from build123d import *

# Parameters (mm, degrees)
SKETCH_1_R                = 810
EXTRUDE_1_DEPTH           = 25
SKETCH_2_R                = 730
EXTRUDE_2_DEPTH           = 5
CUT_EXTRUDE_1_REACH       = 1147.906
SKETCH_3_R                = 75
SKETCH_4_R                = 110
CUT_EXTRUDE_2_DEPTH       = 5
HOLE_WIZARD_M8_1_D        = 6.8
HOLE_WIZARD_25_5_25_5_1_D = 26
CUT_EXTRUDE_3_DEPTH       = 1146.905755287
CUT_EXTRUDE_3_DEPTH_BACK  = 1146.905755287
SKETCH_10_OUTSIDE_W       = 2080.244
SKETCH_10_OUTSIDE_H       = 2080.244
SKETCH_10_OUTSIDE_R       = 675
CHAMFER_1_SIZE            = 10


with BuildPart() as part:
    # 草图1 → 凸台-拉伸1 (new body)
    with BuildSketch(Plane(origin=(0, 0, 0), x_dir=(1, 0, 0), z_dir=(0, 1, 0))):
        with Locations(Location((0, 0, 0), (0, 0, 270))):
            Circle(SKETCH_1_R)
    extrude(amount=EXTRUDE_1_DEPTH)

    # 草图2 → 凸台-拉伸2 (add)
    with BuildSketch(Plane(origin=(0, 25, 0), x_dir=(1, 0, 0), z_dir=(0, 1, 0))):
        with Locations(Location((0, 0, 0), (0, 0, 270))):
            Circle(SKETCH_2_R)
    extrude(amount=EXTRUDE_2_DEPTH)

    # 草图3 → 切除-拉伸1 (cut, up to next)
    with BuildSketch(Plane(origin=(0, 30, 0), x_dir=(1, 0, 0), z_dir=(0, 1, 0)), mode=Mode.PRIVATE) as cut_extrude_1_sk1:
        with BuildLine():
            Line((130, 662.363193422), (130, -662.363193422))
            ThreePointArc((130, -662.363193422), (521.236510617, -428.879353665), (675, 0))
            ThreePointArc((675, 0), (521.236510617, 428.879353665), (130, 662.363193422))
        make_face()
    cut_extrude_1_tool1 = extrude(cut_extrude_1_sk1.sketch, amount=-CUT_EXTRUDE_1_REACH, mode=Mode.PRIVATE) & part.part
    # 草图3 → 切除-拉伸1 (cut, up to next)
    with BuildSketch(Plane(origin=(0, 30, 0), x_dir=(1, 0, 0), z_dir=(0, 1, 0)), mode=Mode.PRIVATE) as cut_extrude_1_sk2:
        with BuildLine():
            ThreePointArc((-130, 662.363193422), (-675, 0), (-130, -662.363193422))
            Line((-130, -662.363193422), (-130, 662.363193422))
        make_face()
    cut_extrude_1_tool2 = extrude(cut_extrude_1_sk2.sketch, amount=-CUT_EXTRUDE_1_REACH, mode=Mode.PRIVATE) & part.part
    # 草图3 → 切除-拉伸1 (cut, up to next)
    with BuildSketch(Plane(origin=(0, 30, 0), x_dir=(1, 0, 0), z_dir=(0, 1, 0)), mode=Mode.PRIVATE) as cut_extrude_1_sk3:
        with Locations(Location((0, 0, 0), (0, 0, 270))):
            Circle(SKETCH_3_R)
    cut_extrude_1_tool3 = extrude(cut_extrude_1_sk3.sketch, amount=-CUT_EXTRUDE_1_REACH, mode=Mode.PRIVATE) & part.part
    add(cut_extrude_1_tool1.solids().sort_by_distance((357.907844, 30, 0))[0], mode=Mode.SUBTRACT)
    add(cut_extrude_1_tool2.solids().sort_by_distance((-357.907844, 30, 0))[0], mode=Mode.SUBTRACT)
    add(cut_extrude_1_tool3.solids().sort_by_distance((0, 30, 0))[0], mode=Mode.SUBTRACT)

    # 草图4 → 切除-拉伸2 (cut)
    with BuildSketch(Plane(origin=(0, 30, 0), x_dir=(1, 0, 0), z_dir=(0, 1, 0))):
        with Locations(Location((0, 0, 0), (0, 0, 270))):
            Circle(SKETCH_4_R)
    extrude(amount=-CUT_EXTRUDE_2_DEPTH, mode=Mode.SUBTRACT)

    # M8 螺纹孔1 (through all)
    with Locations(Plane(origin=(0, 25, 0), x_dir=(1, 0, 0), z_dir=(0, 1, 0))):
        with Locations((0, 85), (85, 0), (0, -85), (-85, 0)):
            Hole(HOLE_WIZARD_M8_1_D / 2)

    # Ø25.5 (25.5) 直径孔1 (through all)
    with Locations(Plane(origin=(0, 25, 0), x_dir=(1, 0, 0), z_dir=(0, 1, 0))):
        with Locations((-59.354305918, 754.167962969), (59.354305918, 754.167962969), (176.601417757, 735.597844781), (289.500016584, 698.914866345), (395.270164208, 645.022284334), (491.307448562, 575.247112976), (575.247112976, 491.307448562), (645.022284334, 395.270164208), (698.914866345, 289.500016584), (735.597844781, 176.601417757), (754.167962969, 59.354305918), (754.167962969, -59.354305918), (735.597844781, -176.601417757), (698.914866345, -289.500016584), (645.022284334, -395.270164208), (575.247112976, -491.307448562), (491.307448562, -575.247112976), (395.270164208, -645.022284334), (289.500016584, -698.914866345), (176.601417757, -735.597844781), (59.354305918, -754.167962969), (-59.354305918, -754.167962969), (-176.601417757, -735.597844781), (-289.500016584, -698.914866345), (-395.270164208, -645.022284334), (-491.307448562, -575.247112976), (-575.247112976, -491.307448562), (-645.022284334, -395.270164208), (-698.914866345, -289.500016584), (-735.597844781, -176.601417757), (-754.167962969, -59.354305918), (-754.167962969, 59.354305918), (-735.597844781, 176.601417757), (-698.914866345, 289.500016584), (-645.022284334, 395.270164208), (-575.247112976, 491.307448562), (-491.307448562, 575.247112976), (-395.270164208, 645.022284334), (-289.500016584, 698.914866345), (-176.601417757, 735.597844781)):
            Hole(HOLE_WIZARD_25_5_25_5_1_D / 2)

    # 草图10 outside → 切除-拉伸3 (cut, two sides: drawn at the far end of the back side and taken through both)
    with BuildSketch(Plane(origin=(0, 30, 0), x_dir=(1, 0, 0), z_dir=(0, 1, 0)).offset(-CUT_EXTRUDE_3_DEPTH_BACK)):
        Rectangle(SKETCH_10_OUTSIDE_W, SKETCH_10_OUTSIDE_H)
        Circle(SKETCH_10_OUTSIDE_R, mode=Mode.SUBTRACT)
    extrude(amount=CUT_EXTRUDE_3_DEPTH + CUT_EXTRUDE_3_DEPTH_BACK, mode=Mode.SUBTRACT)

    # 倒角1
    chamfer_1_edges = [part.edges().sort_by_distance(p)[0] for p in [
        (0, 30, -675),
        (0, 30, 675),
    ]]
    chamfer(chamfer_1_edges, length=CHAMFER_1_SIZE)


solid = part.part
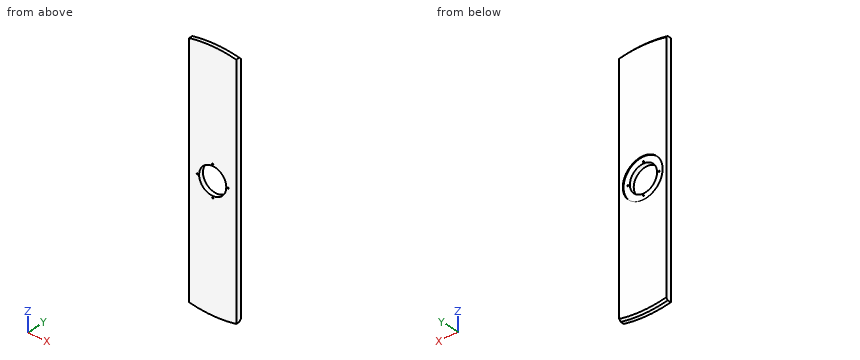
Geometry check sheet. Reference: the model listing, model coordinates, mm. Coordinates: 2 decimals unless noted, no trailing zeros. Order: outer loops, then holes, each group sorted by start corner. A loop starts at its lowest first (then second) coordinate and runs counter-clockwise, first axis right, second up. Notation, with made-up numbers: (70, 53.5) - (117, 53.5) arc R19 cw to (117, 73.5) - close; hole circle Ø3 at (45, 39). An arc over 180 degrees is marked (long way). One line per item, written item: value.
(1) Thickness scan on probe 1 along X at (y, z) = (17.5, -85); probe 2 along Z at (x, y) = (-21, 13.25); probe 3 along Z at (x, y) = (-39, 11). Record the ranges inside material, lowest first. Write a range as from..to.
Data:
probe 1: x = -130..-3.4, 3.4..130
probe 2: z = -674.67..-72, 72..674.67
probe 3: z = -673.87..-64.06, 64.06..673.87
(2) Depth check by flat-ended pin: pin 1 Ø1 at (x, z) = (-96, 71) entering from -Y; pin 2 Ø2 at (x, y) = (97, 16) entering from -Z; pin 3 Ø2 at (x, y) = (90.5, 20.5) entering from -Z; pin 4 Ø12 at (x, y) = (77.5, 26) entering from -Z. Enter the tip coordinate at first touch or a pass-through.
Data:
pin 1: stops at y = 0
pin 2: stops at z = -668.14
pin 3: stops at z = -669.02
pin 4: stops at z = -670.58
(3) Sectioned sample at A-A (z = -56). Enter the section's corners in (x, y).
Data:
outline: (-130, 0) - (-49.89, 0) - (-49.89, 25) - (-94.68, 25) - (-94.68, 30) - (-130, 30) - close; (49.89, 0) - (130, 0) - (130, 30) - (94.68, 30) - (94.68, 25) - (49.89, 25) - close
